from build123d import *

# Parameters (mm, degrees)
SKETCH1_W           = 50
SKETCH1_H           = 150
BOSS_EXTRUDE1_DEPTH = 10
SKETCH2_W           = 30
SKETCH2_H           = 30
CUT_EXTRUDE1_DEPTH  = 10
SKETCH3_R           = 4
CUT_EXTRUDE2_DEPTH  = 80.686887253


with BuildPart() as part:
    # Sketch1 → Boss-Extrude1 (new body)
    with BuildSketch(Plane.XY):
        Rectangle(SKETCH1_W, SKETCH1_H)
    extrude(amount=BOSS_EXTRUDE1_DEPTH)

    # Sketch2 → Cut-Extrude1 (cut)
    with BuildSketch(Plane.XY.offset(10)):
        with Locations((0, 60)):
            Rectangle(SKETCH2_W, SKETCH2_H)
    extrude(amount=-CUT_EXTRUDE1_DEPTH, mode=Mode.SUBTRACT)

    # Sketch3 → Cut-Extrude2 (cut, through all)
    with BuildSketch(Plane.XY.offset(10)):
        with Locations((-14, 5)):
            Circle(SKETCH3_R)
        with Locations(Location((14, 5, 0), (0, 0, 180))):
            Circle(SKETCH3_R)
    extrude(amount=-CUT_EXTRUDE2_DEPTH, mode=Mode.SUBTRACT)


solid = part.part
Read the model definition and answer for the solid it produces. Units are mm, in the model's axes. A direction names the side the tool comes from. Coordinates: 2 decimals unless noted, no trailing zeros. Loops run counter-clockwise (first coordinate to the right, second up) from the corner with the lowest first, then second, coordinate; pieces in that order, holes last.
Q1. This flat-tipped pin is pushed along its axis until it touches: pin 1 Ø1 at (x, z) = (-4, 3.5) entering from +Y. Where does it stop, or does it pass through?
Q2. The part is cut by section A-A on y = 51.5. Write down the section's boundary in (x, z), and give its area (3 significant figures).
Q3. The mould has two halves that part along Y. Classify faces 1 (the face through (-25, -1, 5)), 2 (the face through (-17.2, 2.6, 5.1)), 3 (the face through (-20, 75, 5)), 4 (the face through (0, -75, 5)): +Y half, -Y half, draft (parallel to the pull), parting line (faces both ways), or undercut.
Q4. The part is cut by section C-C on y = 5. Write down the section's boundary in (x, z), and give its area (3 significant figures).
Q5. Which of the six approach directions +Z, -Z, +X, -X, +Y, -Y give full straight-line access (tool end or side, diameter ignored) to faces 5 (the face through (15, 60, 5)), 6 (the face through (18, 5, 5))?
Q6. The part is cut by section B-B on z = 7.75. Write down the section's boundary in (x, y), and give its area (3 significant figures).
Q7. Consider probe 1 along Y at (x, z) = (14, 6); probe 2 along X at (y, z) = (65, 6); probe 3 along X at (y, z) = (7.5, 9). Determine where each line is inside the solid, lowest interval first.
Results below:
1. pin 1: stops at y = 45
2. outline: (-25, 0) - (-15, 0) - (-15, 10) - (-25, 10) - close; (15, 0) - (25, 0) - (25, 10) - (15, 10) - close
2. area: 200 mm2
3. face 1: draft
3. face 2: undercut
3. face 3: +Y half
3. face 4: -Y half
4. outline: (-25, 0) - (-18, 0) - (-18, 10) - (-25, 10) - close; (-10, 0) - (10, 0) - (10, 10) - (-10, 10) - close; (18, 0) - (25, 0) - (25, 10) - (18, 10) - close
4. area: 340 mm2
5. face 5: +Z, -Z, +Y
5. face 6: +Z, -Z
6. outline: (-25, -75) - (25, -75) - (25, 75) - (15, 75) - (15, 45) - (-15, 45) - (-15, 75) - (-25, 75) - close; hole circle Ø8 at (-14, 5); hole circle Ø8 at (14, 5)
6. area: 6,500 mm2
7. probe 1: y = -75 to 1, 9 to 45
7. probe 2: x = -25 to -15, 15 to 25
7. probe 3: x = -25 to -17.12, -10.88 to 10.88, 17.12 to 25
